Job drawing, mm, ordinate dimensions from the low corner. One solid piece. A direction names the side the tool comes from. Round coordinates to 2 decimals unless told otherwise and drop trailing zeros. Loops run counter-clockwise (first coordinate to the right, second up) from the corner with the lowest first, then second, coordinate; pieces in that order, holes last.
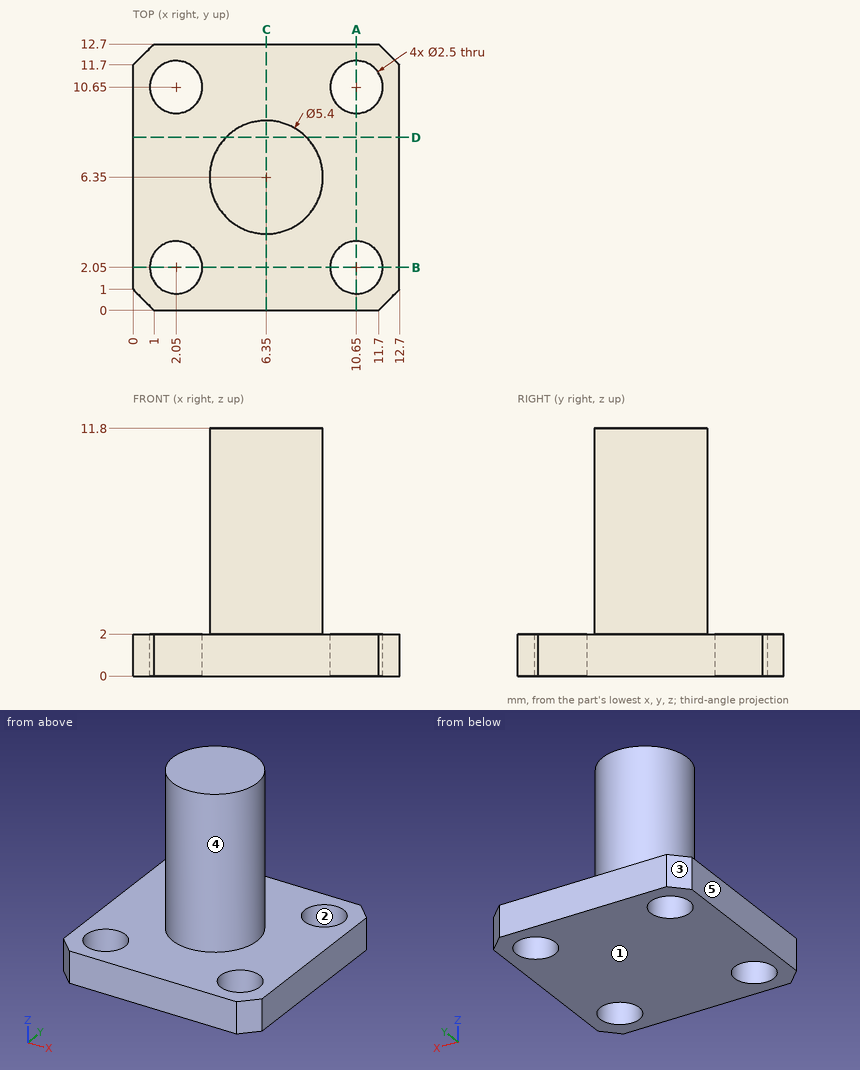
Item 1: Cut at C-C, the plane x = 6.35. Give the cut face in (y, z).
Answers follow:
outline: (0, 0) - (12.7, 0) - (12.7, 2) - (9.05, 2) - (9.05, 11.8) - (3.65, 11.8) - (3.65, 2) - (0, 2) - close
Item 2: Two-plate mould, pull along X, no slides. Class the marked faces 1, 2 and 3: released by +X, released by -X, zero draft, split by the parting line, or undercut.
Answers follow:
face 1: zero draft
face 2: undercut
face 3: released by -X
Item 3: Cut at D-D, the plane y = 8.25. Give the cut face in (x, z).
Answers follow:
outline: (0, 0) - (12.7, 0) - (12.7, 2) - (8.27, 2) - (8.27, 11.8) - (4.43, 11.8) - (4.43, 2) - (0, 2) - close
Item 4: Probe line 1 (Y direction, x = 10.65, z = 0.95); line 2 (Z direction, x = 3.5, y = 8.75). List the from-to ranges inside material, lowest first.
Answers follow:
line 1: y = 0 to 0.8, 3.3 to 9.4, 11.9 to 12.7
line 2: z = 0 to 2
Item 5: 3-axis set-ups, long thin cutter, end or side, ignore diameter. For the marked faces 4 and 5: which of +Z, -Z, +X, -X, +Y, -Y reach the whole face in a straight line?
Answers follow:
face 4: +Z
face 5: +Z, -Z, -X, +Y, -Y
Item 6: Flat gauge pins, fed straight in: P1, Ø3, axis at x = 2.05, y = 10.65, coming from the +Z side; P2, Ø3, axis at y = 7, z = 10, coming from the +X side; P3, Ø2, axis at x = 10.65, y = 10.65, coming from the +Z side; P4, Ø3, axis at x = 5, z = 9, coming from the -Y side. Where does each tip first touch, or does it go through?
Answers follow:
P1: stops at z = 2
P2: stops at x = 9.05
P3: passes through
P4: stops at y = 3.65
Item 7: Cut at A-A, the plane x = 10.65. Give the cut face in (y, z), plus the area to 3 significant figures.
Answers follow:
outline: (0, 0) - (0.8, 0) - (0.8, 2) - (0, 2) - close; (3.3, 0) - (9.4, 0) - (9.4, 2) - (3.3, 2) - close; (11.9, 0) - (12.7, 0) - (12.7, 2) - (11.9, 2) - close
area: 15.4 mm2
